Can you work these out from the model? Positions are in its coordinate system, mm. A direction names the side the tool comes from. Round coordinates to 2 decimals unless told otherwise and drop trailing zeros. Loops run counter-clockwise (first coordinate to the right, second up) from the corner with the lowest first, then second, coordinate; pieces in that order, holes last. Notation, with made-up numbers: (42.25, 23) -> (96.25, 23) arc R24 ccw to (96.25, 49) -> close; hole circle Ø5 at (38, 30.25). An arc over 180 degrees is marked (long way). Write each question's results on one line, items separated by ' | '.
from build123d import *

# Parameters (mm, degrees)
SKETCH1_W           = 300
SKETCH1_H           = 170
BOSS_EXTRUDE1_DEPTH = 10
SKETCH2_W           = 300
SKETCH2_H           = 10
BOSS_EXTRUDE2_DEPTH = 20
SKETCH4_W           = 300
SKETCH4_H           = 10
BOSS_EXTRUDE3_DEPTH = 25
BOSS_EXTRUDE4_DEPTH = 85
CUT_EXTRUDE1_DEPTH  = 15
SKETCH8_R           = 10
BOSS_EXTRUDE5_DEPTH = 15


with BuildPart() as part:
    # Sketch1 → Boss-Extrude1 (new body)
    with BuildSketch(Plane.XY):
        Rectangle(SKETCH1_W, SKETCH1_H)
    extrude(amount=BOSS_EXTRUDE1_DEPTH)

    # Sketch2 → Boss-Extrude2 (add)
    with BuildSketch(Plane.XY.offset(10)):
        with Locations((0, 80)):
            Rectangle(SKETCH2_W, SKETCH2_H)
        with Locations((0, -80)):
            Rectangle(SKETCH2_W, SKETCH2_H)
    extrude(amount=BOSS_EXTRUDE2_DEPTH)

    # Sketch4 → Boss-Extrude3 (add)
    with BuildSketch(Plane.XZ.offset(-75)):
        with Locations((0, 25)):
            Rectangle(SKETCH4_W, SKETCH4_H)
    boss_extrude3 = extrude(amount=BOSS_EXTRUDE3_DEPTH)

    # Mirror1: Boss-Extrude3 across plane
    add(boss_extrude3.mirror(Plane.ZX))

    # Sketch5 → Boss-Extrude4 (add, symmetric)
    with BuildSketch(Plane(origin=(0, 0, 0), x_dir=(1, 0, 0), z_dir=(0, 1, 0))):
        Polygon((-150, 0), (-150, 70), (-135, 70), (-25, 20), (0, 20), (0, 0), align=None)
    boss_extrude4 = extrude(amount=BOSS_EXTRUDE4_DEPTH, both=True)

    # Sketch6 → Cut-Extrude1 (cut, symmetric)
    with BuildSketch(Plane(origin=(0, 0, 0), x_dir=(1, 0, 0), z_dir=(0, 1, 0))):
        Polygon((-150, 70), (-135, 70), (-25, 20), (0, 20), (0, 0), (-25, 0), (-135, 50), (-150, 50), align=None)
    cut_extrude1 = extrude(amount=CUT_EXTRUDE1_DEPTH, both=True, mode=Mode.SUBTRACT)

    # Mirror2: Boss-Extrude4, Cut-Extrude1 across plane
    add(boss_extrude4.mirror(Plane(origin=(0, 0, 0), x_dir=(0, 0, 1), z_dir=(1, 0, 0))))
    add(cut_extrude1.mirror(Plane(origin=(0, 0, 0), x_dir=(0, 0, 1), z_dir=(1, 0, 0))), mode=Mode.SUBTRACT)

    # Sketch8 → Boss-Extrude5 (add, symmetric)
    with BuildSketch(Plane(origin=(0, 0, 0), x_dir=(1, 0, 0), z_dir=(0, 1, 0))):
        with BuildLine():
            Line((150, -6), (190, -6))
            ThreePointArc((190, -6), (215.5, 19.5), (190, 45))
            Line((190, 45), (150, 45))
            Line((150, 45), (150, -6))
        make_face()
        with Locations(Location((190, 19.5, 0), (0, 0, 270))):
            Circle(SKETCH8_R, mode=Mode.SUBTRACT)
    extrude(amount=BOSS_EXTRUDE5_DEPTH, both=True)


solid = part.part
1. If we section it at C-C (x = 124): List the corners of the cut face in (y, z) for me, then the cut area to 4 significant figures.
Final values:
outline: (-85, -65) -> (-15, -65) -> (-15, -45) -> (15, -45) -> (15, -65) -> (85, -65) -> (85, 30) -> (50, 30) -> (50, 20) -> (75, 20) -> (75, 10) -> (-75, 10) -> (-75, 20) -> (-50, 20) -> (-50, 30) -> (-85, 30) -> close | area: 13,050 mm2
2. On a 3-axis mill with a long thin cutter (end or side, diameter ignored), from which of +Z, -Z, +X, -X, +Y, -Y can I reach the whole of each face in a straight line? I mean faces 4 (the face through (-2, -75, 15)), 5 (the face through (80.77, 50.49, -45.35)), 6 (the face through (170, 0, 6)), 7 (the face through (175, -15, -20)). Say none if no direction works.
Final values:
face 4: +X, -X | face 5: -Z, +Y, -Y | face 6: +Z, +X, +Y, -Y | face 7: +Z, -Z, +X, -Y
3. If we section it at B-B (y = -6): List the corners of the cut face in (x, z) for me, then the cut area to 3 significant figures.
Final values:
outline: (-150, -50) -> (-135, -50) -> (-25, 0) -> (25, 0) -> (135, -50) -> (150, -50) -> (150, -45) -> (190, -45) arc R25.5 ccw to (190, 6) -> (150, 6) -> (150, 10) -> (-150, 10) -> close; hole circle Ø20 at (190, -19.5) | area: 12,700 mm2
4. We'd pull the mould along Y, two halves only. Please class faces 1 (the face through (-2, -85, -10)), 2 (the face through (-2, -50, 25)), 3 (the face through (0, -50, -20)): pulls with the +Y half, pulls with the -Y half, needs draft (parallel to the pull), parting line crosses it, or undercut.
Final values:
face 1: pulls with the -Y half | face 2: undercut | face 3: needs draft
5. Please list where these lines run through material, in increasing order: line 1 (X direction, y = -2, z = -19); line 2 (Y direction, x = 112, z = -58); line 3 (X direction, y = 35.5, z = -7). Write a range as from..to.
Final values:
line 1: -150..-66.8, 66.8..180.01, 199.99..215.5 | line 2: -85..-15, 15..85 | line 3: -150..150
6. If we section it at A-A (z = -25.5): List the corners of the cut face in (x, y) for me.
Final values:
outline: (-150, -85) -> (-37.1, -85) -> (-37.1, -15) -> (-81.1, -15) -> (-81.1, 15) -> (-37.1, 15) -> (-37.1, 85) -> (-150, 85) -> close; (37.1, -85) -> (150, -85) -> (150, -15) -> (182, -15) -> (182, 15) -> (150, 15) -> (150, 85) -> (37.1, 85) -> (37.1, 15) -> (81.1, 15) -> (81.1, -15) -> (37.1, -15) -> close; (198, -15) -> (214.78, -15) -> (214.78, 15) -> (198, 15) -> close
7. If we section it at D-D (y = -29): List the corners of the cut face in (x, z) for me, then the cut area to 3 significant figures.
Final values:
outline: (-150, -70) -> (-135, -70) -> (-25, -20) -> (25, -20) -> (135, -70) -> (150, -70) -> (150, 10) -> (-150, 10) -> close | area: 16,000 mm2
8. Will these pins go through, and if not, where does the flat tip stop? pin 1 (8 mm diameter, centred on y = 34.5, z = -27, fed in from +X); pin 2 (7.5 mm diameter, centred on x = 20.5, y = -57.5, fed in from -Z); pin 3 (9 mm diameter, centred on x = 171.5, y = 1, fed in from +Z); pin 4 (18 mm diameter, centred on x = 190, z = -19.5, fed in from -Y).
Final values:
pin 1: x = 150 | pin 2: z = -20 | pin 3: z = 6 | pin 4: through
